Here's how the part is built. I have some questions about the finished solid (model axes, mm). Face numbers are marked on the shaded views. A direction names the side the tool comes from. Coordinates: 2 decimals unless noted, no trailing zeros. Write each loop counter-clockwise with the first axis right and the second up, starting at its lowest first coordinate (ties: lowest second). Pieces come first, ordered by that corner, then holes.
Item 1: I'm going to push flat-ended pins straight in: P1, Ø3, axis at y = 1, z = 12, coming from the -X side; P2, Ø4, axis at x = 6, y = 10, coming from the -Z side. Where does each tip first touch, or does it pass through?
Item 2: I want a section at A-A (x = 0). Please give me the cut outline in (y, z), and give its area (3 significant figures).
Item 3: Please list where these lines run through material, in increasing order: line 1 (Y direction, x = 22.5, z = -14.5); line 2 (Z direction, x = 7, y = 1); line 3 (Z direction, x = -9.5, y = 8.25).
Item 4: I want a section at B-B (z = 0). Please give me the cut outline in (x, y), and give its area (3 significant figures).
Item 5: I want a section at C-C (y = 8). Please give me the cut outline in (x, z), and give its area (3 significant figures).
Item 6: For the marked faces 1 and 2, which set-ups out of +Z, -Z, +X, -X, +Y, -Y let a thin tool reach every point of the face, with its end or its side?
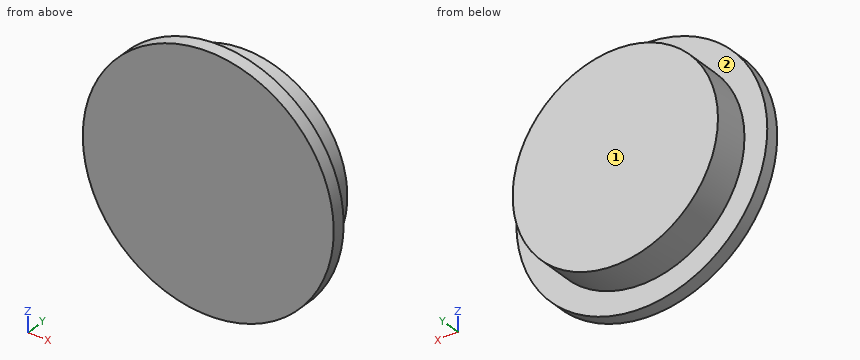
from build123d import *
from build123d.topology import SkipClean

# Parameters (mm, degrees)
REVOLVE_1_ANGLE           = 180
REVOLVE_1_OTHER_WAY_ANGLE = 180


with BuildPart() as part:
    # 草图1 → 旋转1 (revolve)
    with BuildSketch(Plane.XY):
        Polygon((0, 0), (-27.5, 0), (-27.5, 3), (-22.5, 3), (-22.5, 11), (0, 11), align=None)
    revolve(axis=Axis((0, 0, 0), (0, 1, 0)), revolution_arc=REVOLVE_1_ANGLE)

    # 草图1 → 旋转1 other way (revolve)
    with SkipClean():  # the faces are left unmerged after this step: merging them gives an invalid solid
        with BuildSketch(Plane.XY):
            Polygon((0, 0), (-27.5, 0), (-27.5, 3), (-22.5, 3), (-22.5, 11), (0, 11), align=None)
        revolve(axis=Axis((0, 0, 0), (0, -1, 0)), revolution_arc=REVOLVE_1_OTHER_WAY_ANGLE)


solid = part.part
Answer:
1. P1: stops at x = -25.42
1. P2: stops at z = -22.14
2. outline: (0, -27.5) - (3, -27.5) - (3, -22.5) - (11, -22.5) - (11, 22.5) - (3, 22.5) - (3, 27.5) - (0, 27.5) - close
2. area: 525 mm2
3. line 1: y = 0 to 3
3. line 2: z = -26.59 to 26.59
3. line 3: z = -20.4 to 20.4
4. outline: (-27.5, 0) - (27.5, 0) - (27.5, 3) - (22.5, 3) - (22.5, 11) - (-22.5, 11) - (-22.5, 3) - (-27.5, 3) - close
4. area: 525 mm2
5. outline: circle Ø45 at (0, 0)
5. area: 1,590 mm2
6. face 1: +Z, -Z, +X, -X, +Y
6. face 2: +Y
